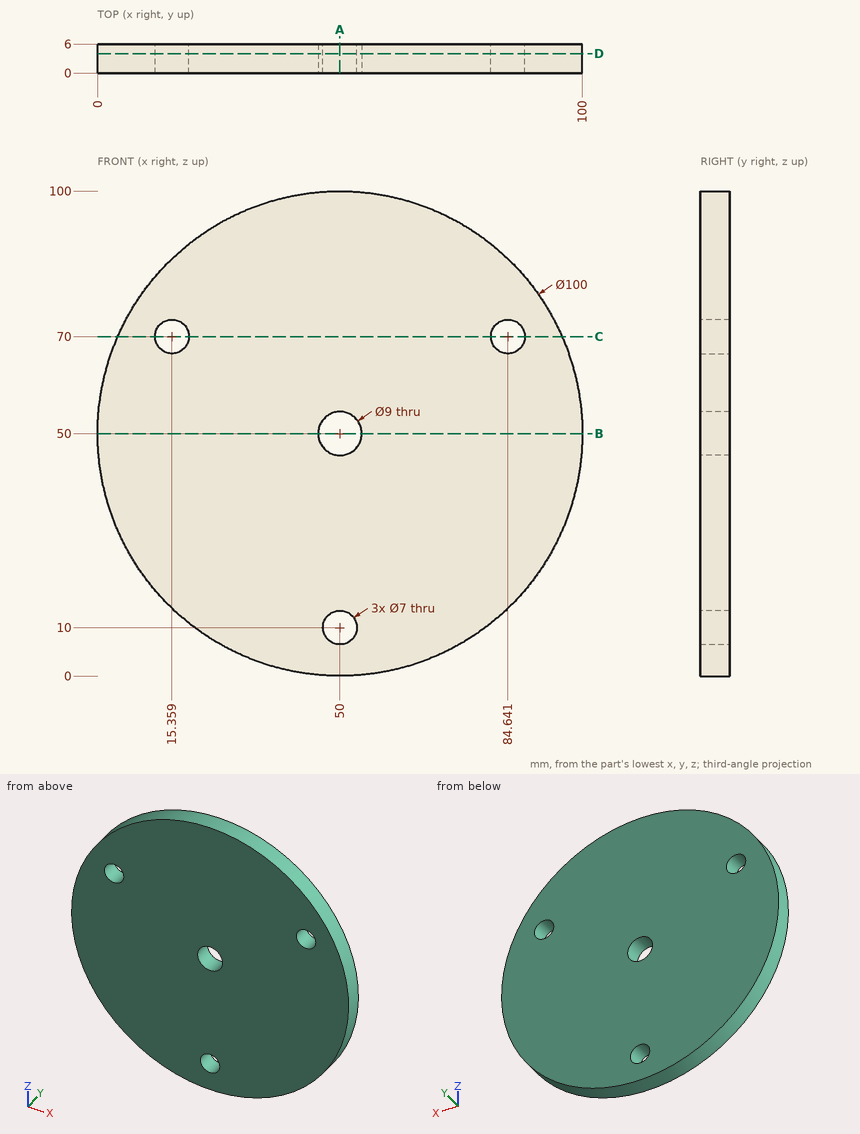
Input: dimensioned drawing with shaded views. Units: mm. Origin: part minimum x, y, z. Coordinates: 2 decimals unless noted, no trailing zeros. Order: outer loops, then holes, each group sorted by start corner. A loop starts at its lowest first (then second) coordinate and runs counter-clockwise, first axis right, second up.
(1) Material intervals for probe 1 along Z at (x, y) = (52.5, 5); probe 2 along X at (y, z) = (1.3, 70); probe 3 along X at (y, z) = (1.7, 50), sorted ascending.
(2) Section query B-B (z = 50). Return the cut outline in (x, y), plus the area to 3 significant figures.
(3) First-contact query: pin 1 (2 mm diameter, centred on y = 3.5, z = 49, fed in from -X); pin 2 (1 mm diameter, centred on y = 3, z = 46, fed in from +X); pin 3 (1 mm diameter, centred on x = 24.5, y = 5, fed in from -Z). Flat tips, straight axial feed; report the tip coordinate or a pass-through.
(4) Section query D-D (y = 4). Return the cut outline in (x, z), plus the area to 3 significant figures.
(5) Section query C-C (z = 70). Return the cut outline in (x, y), plus the area to 3 significant figures.
(6) Section query A-A (x = 50). Return the cut outline in (y, z), plus the area to 3 significant figures.
Solution:
1. probe 1: z = 0.06 to 7.55, 12.45 to 46.26, 53.74 to 99.94
1. probe 2: x = 4.17 to 11.86, 18.86 to 81.14, 88.14 to 95.83
1. probe 3: x = 0 to 45.5, 54.5 to 100
2. outline: (0, 0) - (45.5, 0) - (45.5, 6) - (0, 6) - close; (54.5, 0) - (100, 0) - (100, 6) - (54.5, 6) - close
2. area: 546 mm2
3. pin 1: stops at x = 0
3. pin 2: stops at x = 99.88
3. pin 3: stops at z = 6.7
4. outline: circle Ø100 at (50, 50); hole circle Ø7 at (15.36, 70); hole circle Ø9 at (50, 50); hole circle Ø7 at (50, 10); hole circle Ø7 at (84.64, 70)
4. area: 7,670 mm2
5. outline: (4.17, 0) - (11.86, 0) - (11.86, 6) - (4.17, 6) - close; (18.86, 0) - (81.14, 0) - (81.14, 6) - (18.86, 6) - close; (88.14, 0) - (95.83, 0) - (95.83, 6) - (88.14, 6) - close
5. area: 466 mm2
6. outline: (0, 0) - (6, 0) - (6, 6.5) - (0, 6.5) - close; (0, 13.5) - (6, 13.5) - (6, 45.5) - (0, 45.5) - close; (0, 54.5) - (6, 54.5) - (6, 100) - (0, 100) - close
6. area: 504 mm2
